Input: part model. Units: mm. Frame: model coordinates. Give positions to 0.01 mm unless a question says otherwise; leave off trailing zeros. Loops run counter-clockwise (first coordinate to the right, second up) from the corner with the lowest first, then second, coordinate; pieces in that order, holes last. Notation, with made-up numbers: (41.25, 11) - (89.25, 11) arc R21 cw to (89.25, 40) - close; hole circle Ø6 at (16.5, -24.75). An arc over 180 degrees is marked (long way). One line per item, written item: value.
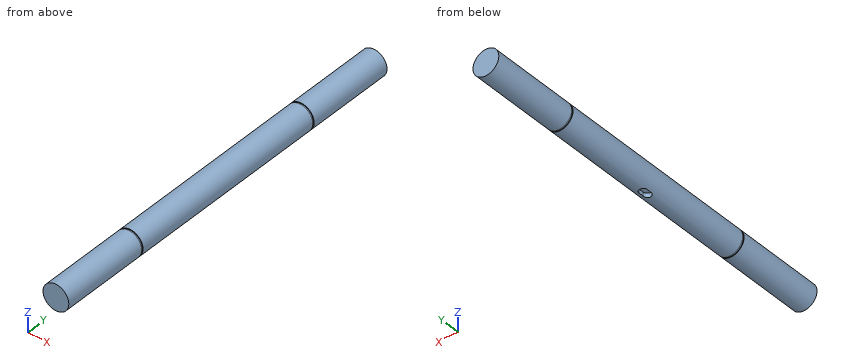
from build123d import *

# Parameters (mm, degrees)
SKETCH_1_R          = 10
EXTRUDE_1_DEPTH     = 300
CUT_EXTRUDE_START   = 1.3
SKETCH_7_R          = 10
SKETCH_7_R_2        = 9.5
CUT_EXTRUDE_3_DEPTH = 1.3
SKETCH_8_R          = 10
SKETCH_8_R_2        = 9.5
CUT_EXTRUDE_4_DEPTH = 1.3
ZJCQC_DEPTH         = 3.5


with BuildPart() as part:
    # 草图1 → 凸台-拉伸1 (new body)
    with BuildSketch(Plane(origin=(0, 0, 0), x_dir=(1, 0, 0), z_dir=(0, 1, 0))):
        with Locations(Location((0, 0, 0), (0, 0, 270))):
            Circle(SKETCH_1_R)
    extrude(amount=EXTRUDE_1_DEPTH)

    # 草图7 → 切除-拉伸3 (cut)
    with BuildSketch(Plane(origin=(0, 70, 0), x_dir=(-1, 0, 0), z_dir=(0, -1, 0)).offset(CUT_EXTRUDE_START)):
        with Locations(Location((0, 0, 0), (0, 0, 90))):
            Circle(SKETCH_7_R)
        with Locations(Location((0, 0, 0), (0, 0, 90))):
            Circle(SKETCH_7_R_2, mode=Mode.SUBTRACT)
    extrude(amount=-CUT_EXTRUDE_3_DEPTH, mode=Mode.SUBTRACT)

    # 草图8 → 切除-拉伸4 (cut)
    with BuildSketch(Plane(origin=(0, 230, 0), x_dir=(1, 0, 0), z_dir=(0, 1, 0))):
        with Locations(Location((0, 0, 0), (0, 0, 90))):
            Circle(SKETCH_8_R)
        with Locations(Location((0, 0, 0), (0, 0, 90))):
            Circle(SKETCH_8_R_2, mode=Mode.SUBTRACT)
    extrude(amount=CUT_EXTRUDE_4_DEPTH, mode=Mode.SUBTRACT)

    # MyToolsZJC → ZJCQC (cut)
    with BuildSketch(Plane.YX.offset(10)):
        with BuildLine():
            Line((148, 3), (152, 3))
            ThreePointArc((152, 3), (155, 0), (152, -3))
            Line((152, -3), (148, -3))
            ThreePointArc((148, -3), (145, 0), (148, 3))
        make_face()
    extrude(amount=-ZJCQC_DEPTH, mode=Mode.SUBTRACT)


solid = part.part
Item 1: Section C-C, the plane y = 23.5. Output: boundary loops of the cut face in (x, z).
Verdict:
outline: circle Ø20 at (0, 0)
Item 2: Section B-B, the plane z = -3.25. Output: boundary loops of the cut face in (x, y).
Verdict:
outline: (-9.46, 0) - (9.46, 0) - (9.46, 68.7) - (8.93, 68.7) - (8.93, 70) - (9.46, 70) - (9.46, 230) - (8.93, 230) - (8.93, 231.3) - (9.46, 231.3) - (9.46, 300) - (-9.46, 300) - (-9.46, 231.3) - (-8.93, 231.3) - (-8.93, 230) - (-9.46, 230) - (-9.46, 70) - (-8.93, 70) - (-8.93, 68.7) - (-9.46, 68.7) - close
Item 3: Material intervals for L1, parallel to Y at x = -5.75, z = 7.75; L2, parallel to Z at x = -0.75, y = 114; L3, parallel to Z at x = -3.25, y = 189, sorted ascending.
Verdict:
L1: y = 0 to 68.7, 70 to 230, 231.3 to 300
L2: z = -9.97 to 9.97
L3: z = -9.46 to 9.46
Item 4: Pin query (flat end, axial travel): P1, Ø1.5, axis at y = 56.5, z = 0.5, coming from the -X side; P2, Ø2, axis at y = 263, z = 4.5, coming from the -X side; P3, Ø1.5, axis at x = -4.5, y = 44.5, coming from the -Z side; P4, Ø6.5, axis at x = 0.5, y = 149, coming from the -Z side. Return the tip coordinate at first contact, or that it passes through.
Verdict:
P1: stops at x = -10
P2: stops at x = -9.37
P3: stops at z = -9.27
P4: stops at z = -9.65
Item 5: Section A-A, the plane x = -6.75. Output: boundary loops of the cut face in (y, z), and give its area (3 significant figures).
Verdict:
outline: (0, -7.38) - (68.7, -7.38) - (68.7, -6.68) - (70, -6.68) - (70, -7.38) - (230, -7.38) - (230, -6.68) - (231.3, -6.68) - (231.3, -7.38) - (300, -7.38) - (300, 7.38) - (231.3, 7.38) - (231.3, 6.68) - (230, 6.68) - (230, 7.38) - (70, 7.38) - (70, 6.68) - (68.7, 6.68) - (68.7, 7.38) - (0, 7.38) - close
area: 4,420 mm^2
